Answer from the drawing. Dimensions are ordinates in mm from the lowest x, y and z of the part. Coordinates: 2 decimals unless noted, no trailing zeros. Order: outer loops, then holes, each group sorted by start corner. A loop starts at its lowest first (then second) coordinate and runs counter-clockwise, first axis right, second up. Notation, with made-up numbers: (2.5, -34.75) -> (45.5, -34.75) arc R23 cw to (45.5, -18.75) -> close; hole circle Ø8 at (-39.5, 67.25). An arc over 180 degrees is marked (long way). Answer in a Markdown table with one row per item.
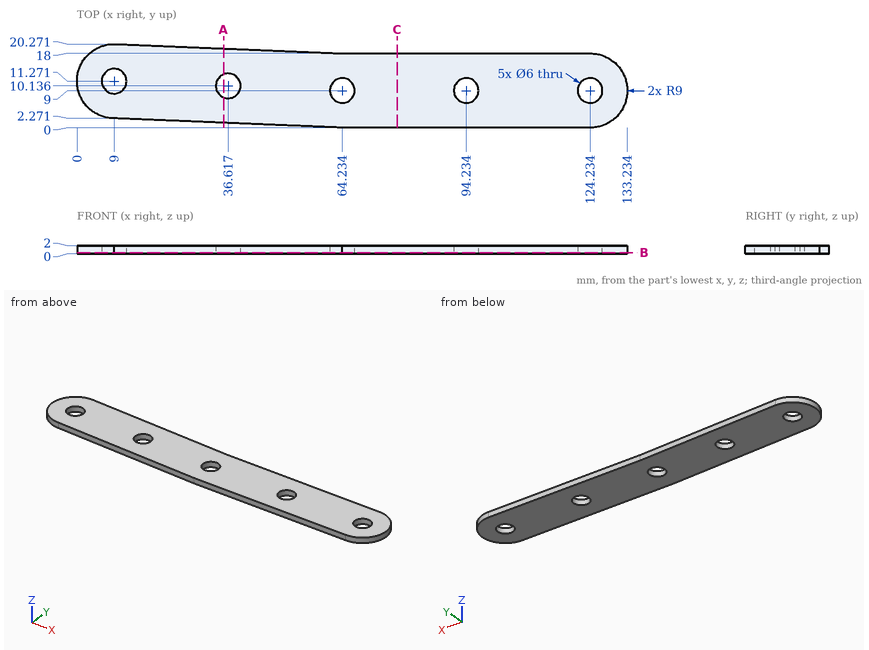
Q1. The part is cut by section A-A (x = 35.5). Write down the section's boundary in (y, z).
Outcome:
| item | result |
|---|---|
| outline | (1.18, 0) -> (7.35, 0) -> (7.35, 2) -> (1.18, 2) -> close; (12.92, 0) -> (19.18, 0) -> (19.18, 2) -> (12.92, 2) -> close |
Q2. The part is cut by section C-C (x = 77.5). Write down the section's boundary in (y, z), then the cut area to 3 significant figures.
Outcome:
| item | result |
|---|---|
| outline | (0, 0) -> (18, 0) -> (18, 2) -> (0, 2) -> close |
| area | 36.0 mm² |
Q3. Consider line 1 (X direction, y = 12.25, z = 0.6) (1 decimal); line 2 (Y direction, x = 9, z = 1.35); line 3 (Y direction, x = 120, z = 1.8). Determine where each line is inside the solid, lowest interval first.
Outcome:
| item | result |
|---|---|
| line 1 | 0.1 to 6.2, 11.8 to 34.5, 38.7 to 132.6 |
| line 2 | 2.27 to 8.27, 14.27 to 20.27 |
| line 3 | 0 to 18 |
Q4. The part is cut by section B-B (z = 0.3). Write down the section's boundary in (x, y) (1 decimal).
Outcome:
| item | result |
|---|---|
| outline | (9, 2.3) -> (64.2, 0) -> (124.2, 0) arc R9 ccw to (124.2, 18) -> (64.2, 18) -> (9, 20.3) arc R9 ccw to start; hole circle Ø6 at (9, 11.3); hole circle Ø6 at (36.6, 10.1); hole circle Ø6 at (64.2, 9); hole circle Ø6 at (94.2, 9); hole circle Ø6 at (124.2, 9) |
Q5. Given pin 1 (0.6 mm diameter, centred on x = 92.5, z = 1.5, fed in from +Y), flat-ended and moving along its own axis, determine where the tip first touches the part or whether it passes through.
Outcome:
| item | result |
|---|---|
| pin 1 | y = 18 |
